Geometry: final body of the model. Coordinates: model frame, mm. Give positions to 0.01 mm unless a question says otherwise; leave off trailing zeros. Write each loop counter-clockwise with the first axis right and the second up, starting at its lowest first coordinate (ties: lowest second). Pieces come first, ordered by that corner, then holes.
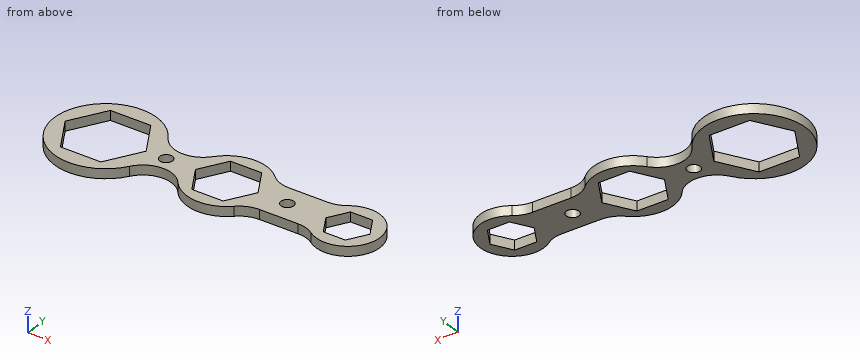
```python
from build123d import *

# Parameters (mm, degrees)
SPANNER_PLATE_6MM_DEPTH        = 6
HEX_OPENINGS_44_34_24_AF_DEPTH = 176.054277297
WEB_HOLES_SKETCH_R             = 4
WEB_HOLES_2X_8_DEPTH           = 176.054277297


with BuildPart() as part:
    # Spanner Outline Sketch → Spanner Plate 6mm (new body)
    with BuildSketch(Plane.XY):
        with BuildLine():
            Line((105.799328852, -13), (130.022739024, -13))
            ThreePointArc((130.022739024, -13), (135.485531832, -13.848968115), (140.433020539, -16.315789474))
            ThreePointArc((140.433020539, -16.315789474), (172, 0), (140.433020539, 16.315789474))
            ThreePointArc((140.433020539, 16.315789474), (135.485531832, 13.848968115), (130.022739024, 13))
            Line((130.022739024, 13), (105.799328852, 13))
            ThreePointArc((105.799328852, 13), (99.075542543, 14.302973388), (93.325191193, 18.023255814))
            ThreePointArc((93.325191193, 18.023255814), (74.306021319, 24.942542698), (56.397031824, 15.515271144))
            ThreePointArc((56.397031824, 15.515271144), (41.324651991, 8.711790831), (27.061052632, 17.079210476))
            ThreePointArc((27.061052632, 17.079210476), (-32, 0), (27.061052632, -17.079210476))
            ThreePointArc((27.061052632, -17.079210476), (41.324651991, -8.711790831), (56.397031824, -15.515271144))
            ThreePointArc((56.397031824, -15.515271144), (74.306021319, -24.942542698), (93.325191193, -18.023255814))
            ThreePointArc((93.325191193, -18.023255814), (99.075542543, -14.302973388), (105.799328852, -13))
        make_face()
    extrude(amount=SPANNER_PLATE_6MM_DEPTH)

    # Hex Openings Sketch → Hex Openings 44-34-24 AF (cut, through all)
    with BuildSketch(Plane.XY.offset(6)):
        Polygon((25.403411844, 0), (12.701705922, 22), (-12.701705922, 22), (-25.403411844, 0), (-12.701705922, -22), (12.701705922, -22), align=None)
        Polygon((95.629909152, 0), (85.814954576, 17), (66.185045424, 17), (56.370090848, 0), (66.185045424, -17), (85.814954576, -17), align=None)
        Polygon((165.856406461, 0), (158.92820323, 12), (145.07179677, 12), (138.143593539, 0), (145.07179677, -12), (158.92820323, -12), align=None)
    extrude(amount=-HEX_OPENINGS_44_34_24_AF_DEPTH, mode=Mode.SUBTRACT)

    # Web Holes Sketch → Web Holes 2xØ8 (cut, through all)
    with BuildSketch(Plane.XY.offset(6)):
        with Locations((38, 0)):
            Circle(WEB_HOLES_SKETCH_R)
        with Locations((114, 0)):
            Circle(WEB_HOLES_SKETCH_R)
    extrude(amount=-WEB_HOLES_2X_8_DEPTH, mode=Mode.SUBTRACT)


solid = part.part
```
Item 1: Pin query (flat end, axial travel): pin 1 Ø10 at (x, y) = (144.5, -13) entering from -Z; pin 2 Ø1.8 at (x, z) = (120, 3.5) entering from -Y; pin 3 Ø3 at (x, z) = (152, 3.5) entering from -Y; pin 4 Ø3 at (x, z) = (-4, 2) entering from +Y. Return the tip coordinate at first contact, or that it passes through.
Found:
pin 1: stops at z = 0
pin 2: stops at y = -13
pin 3: stops at y = -20
pin 4: stops at y = 31.9
Item 2: Section A-A, the plane x = 152. Return the cut outline in (y, z), plus the area to 3 significant figures.
Found:
outline: (-20, 0) - (-12, 0) - (-12, 6) - (-20, 6) - close; (12, 0) - (20, 0) - (20, 6) - (12, 6) - close
area: 96.0 mm2
Item 3: Section B-B, the plane z = 2.85. State how many separate pieces and enclosed holes the cut face has, plus the area to 3 significant figures.
Found:
separate pieces: 1
enclosed holes: 5
area: 4,480 mm2
Item 4: Line query: L1, parallel to Y at x = 114, z = 3.6; L2, parallel to X at y = 4.5, z = 4.1; L3, parallel to X at y = 12.5, z = 2.95. Output: solid intervals per line, ascending.
Found:
L1: y = -13 to -4, 4 to 13
L2: x = -31.68 to -22.81, 22.81 to 58.97, 93.03 to 140.74, 163.26 to 171.49
L3: x = -29.46 to -18.19, 18.19 to 31.2, 53.36 to 63.59, 88.41 to 167.61
Item 5: Section C-C, the plane x = 0. Return the cut outline in (y, z), plus the area to 3 significant figures.
Found:
outline: (-32, 0) - (-22, 0) - (-22, 6) - (-32, 6) - close; (22, 0) - (32, 0) - (32, 6) - (22, 6) - close
area: 120 mm2
